from build123d import *

# Parameters (mm, degrees)
SKETCH_1_W                = 60
SKETCH_1_H                = 20
EXTRUDE_1_DEPTH           = 10
HOLE_WIZARD_1_D           = 5.5
HOLE_WIZARD_1_CBORE_D     = 10
HOLE_WIZARD_1_CBORE_DEPTH = 5.7
HOLE_WIZARD_M5_1_D        = 4.2


with BuildPart() as part:
    # 草图1 → 凸台-拉伸1 (new, symmetric)
    with BuildSketch(Plane(origin=(0, 0, 0), x_dir=(1, 0, 0), z_dir=(0, 1, 0))):
        Rectangle(SKETCH_1_W, SKETCH_1_H)
    extrude(amount=EXTRUDE_1_DEPTH, both=True)

    # 打孔尺寸(%根据)内六角圆柱头螺钉的类型1 (through all)
    with Locations(Plane(origin=(0, 10, 0), x_dir=(1, 0, 0), z_dir=(0, 1, 0))):
        with Locations((20, 0), (-20, 0)):
            CounterBoreHole(HOLE_WIZARD_1_D / 2, HOLE_WIZARD_1_CBORE_D / 2, HOLE_WIZARD_1_CBORE_DEPTH)

    # M5 螺纹孔1 (through all)
    with Locations(Plane.XY.offset(10)):
        with Locations((0, 0)):
            Hole(HOLE_WIZARD_M5_1_D / 2)


solid = part.part
Verification items for the finished model (mm, model axes). A direction names the side the tool comes from. Coordinates: 2 decimals unless noted, no trailing zeros. Order: outer loops, then holes, each group sorted by start corner. A loop starts at its lowest first (then second) coordinate and runs counter-clockwise, first axis right, second up. Notation, with made-up numbers: M 58,-27.5 L 68,-27.5 A12 ccw 68,-22.5 Z; hole C 14,57.25 d11. An arc over 180 degrees is marked long. Return JSON: item names as keys, results as strings.
1) Cross-section at A-A, the plane y = 0. Record the boundary of the cut face in (x, z).
Answer list:
{"outline": "M -30,-10 L -2.1,-10 L -2.1,10 L -30,10 Z; M 2.1,-10 L 30,-10 L 30,10 L 2.1,10 Z; hole C -20,0 d5.5; hole C 20,0 d5.5"}
2) Cross-section at D-D, the plane y = -4. Record the boundary of the cut face in (x, z).
Answer list:
{"outline": "M -30,-10 L 30,-10 L 30,10 L -30,10 Z; hole C -20,0 d5.5; hole C 20,0 d5.5"}
3) Cross-section at B-B, the plane z = 0. Record the boundary of the cut face in (x, y).
Answer list:
{"outline": "M -30,-10 L -22.75,-10 L -22.75,4.3 L -25,4.3 L -25,10 L -30,10 Z; M -17.25,-10 L 17.25,-10 L 17.25,4.3 L 15,4.3 L 15,10 L -15,10 L -15,4.3 L -17.25,4.3 Z; M 22.75,-10 L 30,-10 L 30,10 L 25,10 L 25,4.3 L 22.75,4.3 Z; hole C 0,0 d4.2"}
4) Access from +Z, -Z, +X, -X, +Y, -Y to the whole of each face (thin tool, end or side, straight path). Record for faces 1 (the flat face through (-17.8, 4.3, 2.2)), 2 (the flat face through (-0.4, 2.4, -10)).
Answer list:
{"face 1": "+Y", "face 2": "-Z, +X, -X, +Y, -Y"}
5) Release check for a two-part mould opening along Z. For faces 3 (the flat face through (-0.4, 2.4, 10)), 4 (the cylindrical face through (-2.003, 0.631, -0.14)), 5 (the flat face through (22.2, 4.3, 2.2)) record: +Z half, -Z half, draft (parallel to the pull), parting line (faces both ways), or undercut.
Answer list:
{"face 3": "+Z half", "face 4": "draft", "face 5": "undercut"}
6) Thickness scan on L1, parallel to Z at x = -20, y = 6.25; L2, parallel to X at y = 6, z = -1; L3, parallel to X at y = 0.75, z = 1.25. Record the ranges inside material, lowest first. Write a range as [from, to].
Answer list:
{"L1": "[-10, -5], [5, 10]", "L2": "[-30, -24.9], [-15.1, 15.1], [24.9, 30]", "L3": "[-30, -22.45], [-17.55, -1.96], [1.96, 17.55], [22.45, 30]"}
7) Cross-section at C-C, the plane x = 0. Record the boundary of the cut face in (y, z), and give its area (3 significant figures).
Answer list:
{"outline": "M -10,-10 L -2.1,-10 L -2.1,10 L -10,10 Z; M 2.1,-10 L 10,-10 L 10,10 L 2.1,10 Z", "area": "316 mm2"}
8) Gauge pin test, flat end, axial feed: pin 1 (5 mm diameter, centred on x = -19.5, z = 0.5, fed in from +Y). Record the tip position at first contact, or that the pin passes through.
Answer list:
{"pin 1": "y = 4.3"}
